```python
from build123d import *

# Parameters (mm, degrees)
SKETCH1_W                                = 93
SKETCH1_H                                = 93
BOSS_EXTRUDE1_DEPTH                      = 98
SKETCH2_R                                = 35
CUT_EXTRUDE1_DEPTH                       = 6
SKETCH3_R                                = 30
CUT_EXTRUDE2_DEPTH                       = 114.086250269
CUT_EXTRUDE3_REACH                       = 144.882
CUT_EXTRUDE3_END_RADIUS                  = 30
SKETCH4_W                                = 35
SKETCH4_H                                = 50
FILLET1_R                                = 10
CBORE_FOR_M10_HEX_HEAD_BOLT1_D           = 11
CBORE_FOR_M10_HEX_HEAD_BOLT1_CBORE_D     = 17
CBORE_FOR_M10_HEX_HEAD_BOLT1_CBORE_DEPTH = 78
SKETCH9_R                                = 41
CUT_EXTRUDE4_DEPTH                       = 4
SKETCH10_W                               = 52
SKETCH10_H                               = 50
CUT_EXTRUDE5_DEPTH                       = 3
FILLET2_R                                = 3
M3_TAPPED_HOLE1_D                        = 2.5
M3_TAPPED_HOLE1_DEPTH                    = 7.5
M3_TAPPED_HOLE1_TIP                      = 0.751075774
FILLET3_R                                = 5
CIRPATTERN1_COUNT                        = 4


with BuildPart() as part:
    # Sketch1 → Boss-Extrude1 (new body)
    with BuildSketch(Plane.XY):
        Rectangle(SKETCH1_W, SKETCH1_H)
    extrude(amount=BOSS_EXTRUDE1_DEPTH)

    # Sketch2 → Cut-Extrude1 (cut)
    with BuildSketch(Plane(origin=(0, 0, 0), x_dir=(-1, 0, 0), z_dir=(0, 0, -1))):
        Circle(SKETCH2_R)
    extrude(amount=-CUT_EXTRUDE1_DEPTH, mode=Mode.SUBTRACT)

    # Sketch3 → Cut-Extrude2 (cut, through all)
    with BuildSketch(Plane(origin=(0, 0, 6), x_dir=(-1, 0, 0), z_dir=(0, 0, -1))):
        Circle(SKETCH3_R)
    extrude(amount=-CUT_EXTRUDE2_DEPTH, mode=Mode.SUBTRACT)

    # Cut-Extrude3: up to this cylinder (the profile starts outside it)
    cut_extrude3_end = Plane(origin=(0, 0, 55), z_dir=(0, 0, -1)) * Cylinder(CUT_EXTRUDE3_END_RADIUS, 350.764, mode=Mode.PRIVATE)
    # Sketch4 → Cut-Extrude3 (cut, up to the surface)
    with BuildSketch(Plane(origin=(0, 46.5, 0), x_dir=(1, 0, 0), z_dir=(0, 1, 0)), mode=Mode.PRIVATE) as cut_extrude3_sk1:
        with Locations((0, -55)):
            Rectangle(SKETCH4_W, SKETCH4_H)
    cut_extrude3_tool1 = extrude(cut_extrude3_sk1.sketch, amount=-CUT_EXTRUDE3_REACH, mode=Mode.PRIVATE) - cut_extrude3_end
    add(cut_extrude3_tool1.solids().sort_by_distance((0, 46.5, 55))[0], mode=Mode.SUBTRACT)

    # Fillet1
    fillet1_edges = [part.edges().sort_by_distance(p)[0] for p in [
        (46.5, -46.5, 49),
        (-46.5, -46.5, 49),
        (-46.5, 46.5, 49),
        (46.5, 46.5, 49),
    ]]
    fillet(fillet1_edges, radius=FILLET1_R)

    # CBORE for M10 Hex Head Bolt1 (through all)
    with Locations(Plane.XY.offset(98)):
        with Locations((-36, 36), (36, 36), (36, -36), (-36, -36)):
            CounterBoreHole(CBORE_FOR_M10_HEX_HEAD_BOLT1_D / 2, CBORE_FOR_M10_HEX_HEAD_BOLT1_CBORE_D / 2, CBORE_FOR_M10_HEX_HEAD_BOLT1_CBORE_DEPTH)

    # Sketch9 → Cut-Extrude4 (cut)
    with BuildSketch(Plane.XY.offset(98)):
        Circle(SKETCH9_R)
    extrude(amount=-CUT_EXTRUDE4_DEPTH, mode=Mode.SUBTRACT)

    # Sketch10 → Cut-Extrude5 (cut)
    with BuildSketch(Plane(origin=(0, 46.5, 0), x_dir=(1, 0, 0), z_dir=(0, 1, 0))):
        with Locations((0, -55)):
            Rectangle(SKETCH10_W, SKETCH10_H)
    extrude(amount=-CUT_EXTRUDE5_DEPTH, mode=Mode.SUBTRACT)

    # Fillet2
    fillet2_edges = [part.edges().sort_by_distance(p)[0] for p in [
        (26, 45, 80),
        (-26, 45, 30),
        (26, 45, 30),
        (-26, 45, 80),
    ]]
    fillet(fillet2_edges, radius=FILLET2_R)

    # M3 Tapped Hole1
    with Locations(Plane(origin=(0, 43.5, 0), x_dir=(1, 0, 0), z_dir=(0, 1, 0))):
        with Locations((21, -40), (21, -70), (-21, -70), (-21, -40)):
            Hole(M3_TAPPED_HOLE1_D / 2, depth=M3_TAPPED_HOLE1_DEPTH)
            with Locations((0, 0, -(M3_TAPPED_HOLE1_DEPTH + M3_TAPPED_HOLE1_TIP / 2))):  # 118° drill point
                Cone(0, M3_TAPPED_HOLE1_D / 2, M3_TAPPED_HOLE1_TIP, mode=Mode.SUBTRACT)

    # Fillet3
    fillet3_edges = [part.edges().sort_by_distance(p)[0] for p in [
        (17.5, 33.933492931, 30),
        (17.5, 33.933492931, 80),
        (-17.5, 33.933492931, 80),
        (-17.5, 33.933492931, 30),
    ]]
    fillet(fillet3_edges, radius=FILLET3_R)

    # Sketch14 → M5 Tapped Hole2 (revolve, cut)
    with BuildSketch(Plane(origin=(25, 39, 98), x_dir=(0, -1, 0), z_dir=(1, 0, 0))):
        Polygon((0, 0), (0, 13.6618073), (2.1, 12.4), (2.1, 0), align=None)
    m5_tapped_hole2 = revolve(axis=Axis((25, 39, 104.35), (0, 0, -1)), mode=Mode.SUBTRACT)

    # CirPattern1: M5 Tapped Hole2 ×4 about axis
    cirpattern1_axis = Axis((0, 0, 0), (0, 0, 1))
    for i in range(1, CIRPATTERN1_COUNT):
        add(m5_tapped_hole2.rotate(cirpattern1_axis, i * 360 / CIRPATTERN1_COUNT), mode=Mode.SUBTRACT)


solid = part.part
```
The listing builds one solid part. Answer for the finished solid, in the listing's coordinates (mm). A direction names the side the tool comes from. Coordinates: 2 decimals unless noted, no trailing zeros. Loops run counter-clockwise (first coordinate to the right, second up) from the corner with the lowest first, then second, coordinate; pieces in that order, holes last. Notation, with made-up numbers: (26.25, 73.25) -> (42.25, 73.25) arc R19 ccw to (42.25, 80.25) -> close; hole circle Ø6 at (69, 73.5). An arc over 180 degrees is marked (long way). Return JSON: item names as keys, results as strings. Group by question number.
(1) Determine the mould class of faces 1 (the conical face through (25.36, 39.08, 84.56)), 2 (the flat face through (-22, 43.5, 55)), 3 (the cylindrical face through (-37.84, -44.3, 59.55)) for opening direction Z: released by +Z, released by -Z, zero draft, split by the parting line, or undercut.
(2) Find the intervals of material crossed by probe 1 along Y at (x, z) = (-36, 68); probe 2 along X at (y, z) = (36.5, 28); probe 3 along Z at (x, y) = (21, 38.75), in increasing order. Write a range as from..to.
(3) A cutting plane is placed at B-B on y = 18. Write down the section's boundary in (x, z), and give its area (3 significant figures).
(4) A cutting plane is placed at C-C on x = -6. Write down the section's boundary in (y, z), and give its area (3 significant figures).
(5) A cutting plane is placed at D-D on x = 10.5. Write down the section's boundary in (y, z).
(6) Which of the six approach directions +Z, -Z, +X, -X, +Y, -Y give full straight-line access (tool end or side, diameter ignored) to faces 4 (the flat face through (-1, -46.5, 48)), 5 (the cylindrical face through (34.16, 27.7, 59.55)), 6 (the cylindrical face through (16, 33.8, 31.43))?
(7) Given pin 1 Ø11 at (x, z) = (-18, 63) entering from +Y; pin 2 Ø12 at (x, y) = (-9, -26) entering from +Z; pin 3 Ø8.5 at (x, y) = (-32.5, -38) entering from +Z, each flat-ended and moving along its own axis, determine where each tip first touches the part or whether it passes through.
(8) A cutting plane is placed at A-A on z = 92. Count the separate pieces of the cut face and the enclosed holes in it, and give its area (3 significant figures).
The answers:
{
 "1": {"face 1": "released by +Z", "face 2": "undercut", "face 3": "zero draft"},
 "2": {"probe 1": "y = -46.5..-44.5, -27.5..27.5, 44.5..46.5", "probe 2": "x = -46.5..-44.49, -27.51..27.51, 44.49..46.5", "probe 3": "z = 0..38.75, 41.25..68.75, 71.25..98"},
 "3": {"outline": "(-46.5, 0) -> (-30.02, 0) -> (-30.02, 6) -> (-24, 6) -> (-24, 94) -> (-36.84, 94) -> (-36.84, 98) -> (-46.5, 98) -> close; (24, 6) -> (30.02, 6) -> (30.02, 0) -> (46.5, 0) -> (46.5, 98) -> (36.84, 98) -> (36.84, 94) -> (24, 94) -> close", "area": "4,240 mm^2"},
 "4": {"outline": "(-46.5, 0) -> (-34.48, 0) -> (-34.48, 6) -> (-29.39, 6) -> (-29.39, 94) -> (-40.56, 94) -> (-40.56, 98) -> (-46.5, 98) -> close; (29.39, 6) -> (34.48, 6) -> (34.48, 0) -> (46.5, 0) -> (46.5, 30) -> (29.39, 30) -> close; (29.39, 80) -> (46.5, 80) -> (46.5, 98) -> (40.56, 98) -> (40.56, 94) -> (29.39, 94) -> close", "area": "2,350 mm^2"},
 "5": {"outline": "(-46.5, 0) -> (-33.39, 0) -> (-33.39, 6) -> (-28.1, 6) -> (-28.1, 94) -> (-39.63, 94) -> (-39.63, 98) -> (-46.5, 98) -> close; (28.1, 6) -> (33.39, 6) -> (33.39, 0) -> (46.5, 0) -> (46.5, 30) -> (28.1, 30) -> close; (28.1, 80) -> (46.5, 80) -> (46.5, 98) -> (39.63, 98) -> (39.63, 94) -> (28.1, 94) -> close"},
 "6": {"face 4": "+Z, -Z, +X, -X, -Y", "face 5": "+Z", "face 6": "+Y"},
 "7": {"pin 1": "stops at y = 43.5", "pin 2": "stops at z = 94", "pin 3": "stops at z = 20"},
 "8": {"separate pieces": "1", "enclosed holes": "9", "area": "4,770 mm^2"}
}
